Build history of the part. All positions in model axes, mm. A direction names the side the tool comes from. Coordinates: 2 decimals unless noted, no trailing zeros. Loops run counter-clockwise (first coordinate to the right, second up) from the corner with the lowest first, then second, coordinate; pieces in that order, holes last. Notation, with made-up numbers: (6.5, 52.25) -> (52.5, 52.25) arc R19 cw to (52.5, 80.25) -> close; hole circle Ø8 at (65.25, 87). An arc over 180 degrees is marked (long way). One line per item, written item: value. Start each with the question number.
```python
from build123d import *

# Parameters (mm, degrees)
SKETCH1_W                = 90
SKETCH1_H                = 90
BOSS_EXTRUDE1_DEPTH      = 20
CHAMFER1_SIZE            = 3
M8_TAPPED_HOLE1_D        = 6.8
M8_TAPPED_HOLE1_DEPTH    = 19.75
M8_TAPPED_HOLE1_TIP      = 2.042926105
SKETCH4_W                = 15
SKETCH4_H                = 25
CUT_EXTRUDE1_DEPTH       = 42
FILLET1_R                = 3
CHAMFER2_SIZE            = 3
CIRPATTERN2_COUNT        = 4
FILLET1_OF_CIRPATTERN2_R = 3
CHAMFER3_SIZE            = 3
SKETCH5_W                = 27.5
SKETCH5_H                = 27.5
CUT_EXTRUDE2_DEPTH       = 42
CIRPATTERN3_COUNT        = 4
CHAMFER4_SIZE            = 3
FILLET2_R                = 3
SKETCH6_R                = 5
CUT_EXTRUDE3_DEPTH       = 42
CIRPATTERN4_COUNT        = 4
M8_TAPPED_HOLE2_D        = 6.8
M8_TAPPED_HOLE2_DEPTH    = 19.75
M8_TAPPED_HOLE2_TIP      = 2.042926105


with BuildPart() as part:
    # Sketch1 → Boss-Extrude1 (new body)
    with BuildSketch(Plane(origin=(0, 0, 0), x_dir=(1, 0, 0), z_dir=(0, 1, 0))):
        Rectangle(SKETCH1_W, SKETCH1_H)
    extrude(amount=BOSS_EXTRUDE1_DEPTH)

    # Chamfer1
    chamfer1_edges = [part.edges().sort_by_distance(p)[0] for p in [
        (-45, 10, -45),
        (45, 10, -45),
        (45, 10, 45),
        (-45, 10, 45),
    ]]
    chamfer(chamfer1_edges, length=CHAMFER1_SIZE)

    # M8 Tapped Hole1
    with Locations(Plane(origin=(0, 20, 0), x_dir=(1, 0, 0), z_dir=(0, 1, 0))):
        with Locations((0, 0)):
            Hole(M8_TAPPED_HOLE1_D / 2, depth=M8_TAPPED_HOLE1_DEPTH)
            with Locations((0, 0, -(M8_TAPPED_HOLE1_DEPTH + M8_TAPPED_HOLE1_TIP / 2))):  # 118° drill point
                Cone(0, M8_TAPPED_HOLE1_D / 2, M8_TAPPED_HOLE1_TIP, mode=Mode.SUBTRACT)

    # Sketch4 → Cut-Extrude1 (cut)
    with BuildSketch(Plane(origin=(0, 20, 0), x_dir=(1, 0, 0), z_dir=(0, 1, 0))):
        with Locations((0, 32.5)):
            Rectangle(SKETCH4_W, SKETCH4_H)
    cut_extrude1 = extrude(amount=-CUT_EXTRUDE1_DEPTH, mode=Mode.SUBTRACT)

    # Fillet1
    fillet1_edges = [part.edges().sort_by_distance(p)[0] for p in [
        (7.5, 10, -20),
        (-7.5, 10, -20),
    ]]
    fillet(fillet1_edges, radius=FILLET1_R)

    # Chamfer2
    chamfer2_edges = [part.edges().sort_by_distance(p)[0] for p in [
        (7.5, 10, -45),
        (-7.5, 10, -45),
    ]]
    chamfer(chamfer2_edges, length=CHAMFER2_SIZE)

    # CirPattern2: Cut-Extrude1 ×4 about axis
    cirpattern2_axis = Axis((0, 0, 0), (0, 1, 0))
    for i in range(1, CIRPATTERN2_COUNT):
        add(cut_extrude1.rotate(cirpattern2_axis, i * 360 / CIRPATTERN2_COUNT), mode=Mode.SUBTRACT)

    # Fillet1 of CirPattern2
    fillet1_of_cirpattern2_edges = [part.edges().sort_by_distance(p)[0] for p in [
        (-20, 10, -7.5),
        (-20, 10, 7.5),
        (-7.5, 10, 20),
        (7.5, 10, 20),
        (20, 10, 7.5),
        (20, 10, -7.5),
    ]]
    fillet(fillet1_of_cirpattern2_edges, radius=FILLET1_OF_CIRPATTERN2_R)

    # Chamfer3
    chamfer3_edges = [part.edges().sort_by_distance(p)[0] for p in [
        (-45, 10, -7.5),
        (-45, 10, 7.5),
        (-7.5, 10, 45),
        (7.5, 10, 45),
        (45, 10, 7.5),
        (45, 10, -7.5),
    ]]
    chamfer(chamfer3_edges, length=CHAMFER3_SIZE)

    # Sketch5 → Cut-Extrude2 (cut)
    with BuildSketch(Plane(origin=(0, 20, 0), x_dir=(1, 0, 0), z_dir=(0, 1, 0))):
        with Locations((-31.25, 31.25)):
            Rectangle(SKETCH5_W, SKETCH5_H)
    cut_extrude2 = extrude(amount=-CUT_EXTRUDE2_DEPTH, mode=Mode.SUBTRACT)

    # CirPattern3: Cut-Extrude2 ×4 about axis
    cirpattern3_axis = Axis((0, 0, 0), (0, 1, 0))
    for i in range(1, CIRPATTERN3_COUNT):
        add(cut_extrude2.rotate(cirpattern3_axis, i * 360 / CIRPATTERN3_COUNT), mode=Mode.SUBTRACT)

    # Chamfer4
    chamfer4_edges = [part.edges().sort_by_distance(p)[0] for p in [
        (-17.5, 10, -45),
        (-45, 10, -17.5),
        (-45, 10, 17.5),
        (-17.5, 10, 45),
        (17.5, 10, 45),
        (45, 10, 17.5),
        (45, 10, -17.5),
        (17.5, 10, -45),
    ]]
    chamfer(chamfer4_edges, length=CHAMFER4_SIZE)

    # Fillet2
    fillet2_edges = [part.edges().sort_by_distance(p)[0] for p in [
        (-17.5, 10, -17.5),
        (-17.5, 10, 17.5),
        (17.5, 10, 17.5),
        (17.5, 10, -17.5),
    ]]
    fillet(fillet2_edges, radius=FILLET2_R)

    # Sketch6 → Cut-Extrude3 (cut)
    with BuildSketch(Plane.ZY.offset(17.5)):
        with Locations((-35, 10)):
            Circle(SKETCH6_R)
    cut_extrude3 = extrude(amount=-CUT_EXTRUDE3_DEPTH, mode=Mode.SUBTRACT)

    # CirPattern4: Cut-Extrude3 ×4 about axis
    cirpattern4_axis = Axis((0, 20, 0), (0, 1, 0))
    for i in range(1, CIRPATTERN4_COUNT):
        add(cut_extrude3.rotate(cirpattern4_axis, i * 360 / CIRPATTERN4_COUNT), mode=Mode.SUBTRACT)

    # M8 Tapped Hole2
    with Locations(Plane(origin=(0, 20, 0), x_dir=(1, 0, 0), z_dir=(0, 1, 0))):
        with Locations((-10.606601718, -10.606601718), (10.606601718, 10.606601718)):
            Hole(M8_TAPPED_HOLE2_D / 2, depth=M8_TAPPED_HOLE2_DEPTH)
            with Locations((0, 0, -(M8_TAPPED_HOLE2_DEPTH + M8_TAPPED_HOLE2_TIP / 2))):  # 118° drill point
                Cone(0, M8_TAPPED_HOLE2_D / 2, M8_TAPPED_HOLE2_TIP, mode=Mode.SUBTRACT)


solid = part.part
```
Item 1: Band-saw the part on C-C, the plane z = 35. List the corners of the cut face in (x, y).
Item 2: Tool access for faces 1 (the face through (0, 10, 20)), 2 (the face through (-20.86, 9.86, -6.6)), 3 (the face through (-29, 10, 17.5)), 4 (the face through (-12.18, 9.99, 13.62)), 5 (the face through (-9, 10.1, -43.5)): list every direction of +Z, -Z, +X, -X, +Y, -Y with a clear straight run to the whole face (end or side of a thin tool).
Item 3: Band-saw the part on B-B, the plane z = 0. List the corners of the cut face in (x, y), and give its area (3 significant figures).
Item 4: Band-saw the part on D-D, the plane x = 0. List the corners of the cut face in (y, z).
Item 5: Drop flat-ended pins along their axis: pin 1 Ø1 at (y, z) = (16, 25) entering from -X; pin 2 Ø9.5 at (y, z) = (8, -35.5) entering from +X; pin 3 Ø6 at (x, y) = (28.5, 14) entering from +Z; pin 4 Ø6 at (y, z) = (11, 36.5) entering from -X. Give the stop position or say it passes through.
Item 6: Two-plate mould, pull along X, no slides. Class faces 6 (the face through (30, 12, 7.5)), 7 (the face through (-16, 10.1, 43.5)), 8 (the face through (18.4, 9.86, 18.36)), 9 (the face through (7.5, 12, -30)): +X half, -X half, draft (parallel to the pull), parting line (faces both ways), or undercut.
Item 7: Probe probe 1 along Z at (x, y) = (-10, 14.5); probe 2 along Z at (x, y) = (32, 4.25); probe 3 along Y at (x, z) = (35, 11). List the from-to ranges inside material, lowest first.
Item 8: Band-saw the part on A-A, the plane x = -35. List the corners of the cut face in (y, z).
Worked out:
1. outline: (-17.5, 0) -> (-7.5, 0) -> (-7.5, 5) -> (-17.5, 5) -> close; (-17.5, 15) -> (-7.5, 15) -> (-7.5, 20) -> (-17.5, 20) -> close; (7.5, 0) -> (17.5, 0) -> (17.5, 5) -> (7.5, 5) -> close; (7.5, 15) -> (17.5, 15) -> (17.5, 20) -> (7.5, 20) -> close
2. face 1: +Z, +Y, -Y
2. face 2: -X, +Y, -Y
2. face 3: +Z, -X, +Y, -Y
2. face 4: +Y
2. face 5: -Z, +Y, -Y
3. outline: (-20, 0) -> (-2.98, 0) -> (-3.4, 0.25) -> (-3.4, 20) -> (-20, 20) -> close; (2.98, 0) -> (20, 0) -> (20, 20) -> (3.4, 20) -> (3.4, 0.25) -> close
3. area: 664 mm²
4. outline: (0, -20) -> (20, -20) -> (20, -3.4) -> (0.25, -3.4) -> (0, -2.98) -> close; (0, 2.98) -> (0.25, 3.4) -> (20, 3.4) -> (20, 20) -> (0, 20) -> close
5. pin 1: stops at x = -17.5
5. pin 2: stops at x = 17.5
5. pin 3: stops at z = 17.5
5. pin 4: passes through
6. face 6: draft
6. face 7: -X half
6. face 8: +X half
6. face 9: undercut
7. probe 1: z = -44.5 to -37.18, -32.82 to 7.26, 13.95 to 32.82, 37.18 to 44.5
7. probe 2: z = -17.5 to -7.5, 7.5 to 17.5
7. probe 3: y = 0 to 5, 15 to 20
8. outline: (0, -17.5) -> (5, -17.5) -> (5, -7.5) -> (0, -7.5) -> close; (0, 7.5) -> (5, 7.5) -> (5, 17.5) -> (0, 17.5) -> close; (15, -17.5) -> (20, -17.5) -> (20, -7.5) -> (15, -7.5) -> close; (15, 7.5) -> (20, 7.5) -> (20, 17.5) -> (15, 17.5) -> close
